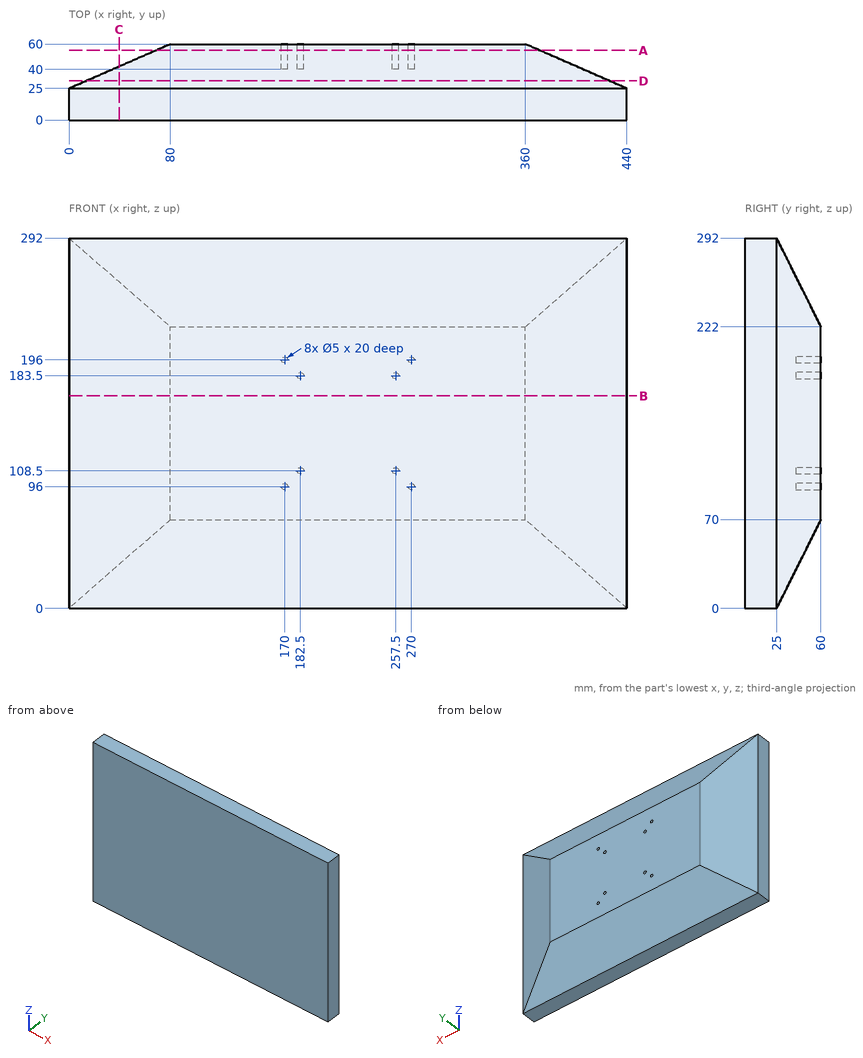
Source: three-view drawing plus pictorial views. Frame: mm from the lowest corner of the part. Give positions to 0.01 mm unless a question says otherwise; leave off trailing zeros. Write each loop counter-clockwise with the first axis right and the second up, starting at its lowest first coordinate (ties: lowest second). Pieces come first, ordered by that corner, then holes. Notation, with made-up numbers: (22, 4) - (61, 4) arc R27 cw to (61, 20) - close; hole circle Ø2 at (-8, 84.25). An arc over 180 degrees is marked (long way). Write item = value, one per line. Start each with the question number.
1. Section query B-B, the plane z = 167.5. Output: boundary loops of the cut face in (x, y), then the cut area to 3 significant figures.
2. Section query A-A, the plane y = 55. Count the separate pieces of the cut face and the enclosed holes in it, then the cut area to 3 significant figures.
3. Section query C-C, the plane x = 39.5. Output: boundary loops of the cut face in (y, z).
4. First-contact query: pin 1 Ø12 at (y, z) = (49, 182.5) entering from +X; pin 2 Ø1.5 at (x, z) = (181.5, 109) entering from +Y; pin 3 Ø8 at (x, y) = (328.5, 39.5) entering from -Z. Flat tips, straight axial feed; report the tip coordinate or a pass-through.
5. Section query D-D, the plane y = 31. Output: boundary loops of the cut face in (x, z).
6. Ray query, L1, parallel to X at y = 45, z = 196; L2, parallel to X at y = 54.75, z = 108.5; L3, parallel to Y at x = 284, z = 262. Return the intervals inside material, ascending.
Check sheet entries:
q1.outline = (0, 0) - (440, 0) - (440, 25) - (360, 60) - (80, 60) - (0, 25) - close
q1.area = 23,600 mm2
q2.separate_pieces = 1
q2.enclosed_holes = 8
q2.area = 51,900 mm2
q3.outline = (0, 0) - (25, 0) - (42.28, 34.56) - (42.28, 257.44) - (25, 292) - (0, 292) - close
q4.pin_1 = 398.86
q4.pin_2 = 40
q4.pin_3 = 21
q5.outline = (13.71, 12) - (426.29, 12) - (426.29, 280) - (13.71, 280) - close
q6.L1 = 45.71 to 167.5, 172.5 to 267.5, 272.5 to 394.29
q6.L2 = 68 to 180, 185 to 255, 260 to 372
q6.L3 = 0 to 40
